For this review, take the finished solid that the model builds, in its own axes (mm). A direction names the side the tool comes from. Give positions to 0.01 mm unless a question says otherwise; leave off trailing zeros. Loops run counter-clockwise (first coordinate to the right, second up) from the corner with the lowest first, then second, coordinate; pieces in that order, holes last.
```python
from build123d import *

# Parameters (mm, degrees)
EXTRUDE_1_DEPTH           = 7.5
SKETCH_2_R                = 11
CUT_EXTRUDE_1_DEPTH       = 6
CUT_EXTRUDE_2_REACH       = 111.663
SKETCH_3_R                = 9.5
CUT_EXTRUDE_3_DEPTH       = 1.5
HOLE_WIZARD_M5_1_D        = 4.2
HOLE_WIZARD_M5_1_DEPTH    = 12.4
HOLE_WIZARD_M5_1_TIP      = 1.2618073
HOLE_WIZARD_1_D           = 5.5
HOLE_WIZARD_1_CBORE_D     = 10
HOLE_WIZARD_1_CBORE_DEPTH = 5.7
HOLE_WIZARD_M3_2_D        = 2.5
CUT_EXTRUDE_START         = -6
SKETCH_17_R               = 11
CUT_EXTRUDE_4_DEPTH       = 6
HOLE_WIZARD_M6_1_D        = 5
HOLE_WIZARD_M6_1_DEPTH    = 15
HOLE_WIZARD_M6_1_TIP      = 1.502151548
CHAMFER_1_SIZE            = 2


with BuildPart() as part:
    # 草图1 → 凸台-拉伸1 (new, symmetric)
    with BuildSketch(Plane(origin=(0, 0, 0), x_dir=(0, 0, -1), z_dir=(1, 0, 0))):
        with BuildLine():
            Line((-10, 101), (-10, 36))
            ThreePointArc((-10, 36), (-12.928932188, 28.928932188), (-20, 26))
            Line((-20, 26), (-40, 26))
            Line((-40, 26), (-40, -101))
            Line((-40, -101), (40, -101))
            Line((40, -101), (40, 101))
            Line((40, 101), (-10, 101))
        make_face()
    extrude(amount=EXTRUDE_1_DEPTH, both=True)

    # 草图2 → 切除-拉伸1 (cut)
    with BuildSketch(Plane.ZY.offset(-7.5)):
        with Locations((-25, 71)):
            Circle(SKETCH_2_R)
    extrude(amount=CUT_EXTRUDE_1_DEPTH, mode=Mode.SUBTRACT)

    # 草图3 → 切除-拉伸2 (cut, up to next)
    with BuildSketch(Plane(origin=(-7.5, 0, 0), x_dir=(0, 0, -1), z_dir=(1, 0, 0)), mode=Mode.PRIVATE) as cut_extrude_2_sk1:
        with Locations(Location((25, 71, 0), (0, 0, 180))):
            Circle(SKETCH_3_R)
    cut_extrude_2_tool1 = extrude(cut_extrude_2_sk1.sketch, amount=CUT_EXTRUDE_2_REACH, mode=Mode.PRIVATE) & part.part
    add(cut_extrude_2_tool1.solids().sort_by_distance((-7.5, 71, -25))[0], mode=Mode.SUBTRACT)

    # 草图6 → 切除-拉伸3 (cut)
    with BuildSketch(Plane(origin=(7.5, 0, 0), x_dir=(0, 0, -1), z_dir=(1, 0, 0))):
        with BuildLine():
            Line((-5.5, 101), (3.5, 101))
            Line((3.5, 101), (3.5, -3.25))
            ThreePointArc((3.5, -3.25), (4.030330086, -4.530330086), (2.75, -4))
            Line((2.75, -4), (-4.75, -4))
            ThreePointArc((-4.75, -4), (-6.030330086, -4.530330086), (-5.5, -3.25))
            Line((-5.5, -3.25), (-5.5, 101))
        make_face()
    extrude(amount=-CUT_EXTRUDE_3_DEPTH, mode=Mode.SUBTRACT)

    # M5 螺纹孔1
    with Locations(Plane(origin=(0, -101, 0), x_dir=(-1, 0, 0), z_dir=(0, -1, 0))):
        with Locations((0, 25), (0, -25)):
            Hole(HOLE_WIZARD_M5_1_D / 2, depth=HOLE_WIZARD_M5_1_DEPTH)
            with Locations((0, 0, -(HOLE_WIZARD_M5_1_DEPTH + HOLE_WIZARD_M5_1_TIP / 2))):  # 118° drill point
                Cone(0, HOLE_WIZARD_M5_1_D / 2, HOLE_WIZARD_M5_1_TIP, mode=Mode.SUBTRACT)

    # 打孔尺寸(%根据)内六角圆柱头螺钉的类型1 (through all)
    with Locations(Plane(origin=(7.5, 0, 0), x_dir=(0, 0, -1), z_dir=(1, 0, 0))):
        with Locations((30, 4), (-30, 4)):
            CounterBoreHole(HOLE_WIZARD_1_D / 2, HOLE_WIZARD_1_CBORE_D / 2, HOLE_WIZARD_1_CBORE_DEPTH)

    # M3 螺纹孔2 (through all)
    with Locations(Plane(origin=(6, 0, 0), x_dir=(0, 0, -1), z_dir=(1, 0, 0))):
        with Locations((-1, 91), (-1, 71), (-1, 51), (-1, 31), (-1, 11)):
            Hole(HOLE_WIZARD_M3_2_D / 2)

    # 草图17 → 切除-拉伸4 (cut)
    with BuildSketch(Plane.ZY.offset(7.5).offset(CUT_EXTRUDE_START)):
        with Locations((-25, 71)):
            Circle(SKETCH_17_R)
    extrude(amount=CUT_EXTRUDE_4_DEPTH, mode=Mode.SUBTRACT)

    # M6 螺纹孔1
    with Locations(Plane(origin=(0, 0, -40), x_dir=(-1, 0, 0), z_dir=(0, 0, -1))):
        with Locations((0, 51), (0, 91)):
            Hole(HOLE_WIZARD_M6_1_D / 2, depth=HOLE_WIZARD_M6_1_DEPTH)
            with Locations((0, 0, -(HOLE_WIZARD_M6_1_DEPTH + HOLE_WIZARD_M6_1_TIP / 2))):  # 118° drill point
                Cone(0, HOLE_WIZARD_M6_1_D / 2, HOLE_WIZARD_M6_1_TIP, mode=Mode.SUBTRACT)

    # 倒角1
    chamfer_1_edges = [part.edges().sort_by_distance(p)[0] for p in [
        (0, 26, 40),
        (0, 101, 10),
        (0, 101, -40),
    ]]
    chamfer(chamfer_1_edges, length=CHAMFER_1_SIZE)


solid = part.part
```
Item 1: Tool access review of faces 1 (the cylindrical face through (5, 4, -25)), 2 (the cylindrical face through (1.13, -94.71, -26.77)), 3 (the cylindrical face through (-0.33, 93.48, -32.39)): name each direction out of +Z, -Z, +X, -X, +Y, -Y from which nothing blocks a thin tool from reaching the whole face with its end or side.
Answer:
face 1: +X
face 2: -Y
face 3: -Z
Item 2: For L1, parallel to Z at x = 0, y = -93.5; L2, parallel to Y at x = 2.75, z = 1; L3, parallel to X at y = 51, z = -30.75, list the stretches that pass through material, from the lowest coordinate up.
Answer:
L1: z = -40 to -27.1, -22.9 to 22.9, 27.1 to 40
L2: y = -101 to 9.75, 12.25 to 29.75, 32.25 to 49.75, 52.25 to 69.75, 72.25 to 89.75, 92.25 to 101
L3: x = -7.5 to -2.5, 2.5 to 7.5
Item 3: Take a section at C-C on y = 45. Give the boundary of the cut face in (x, z), and give its area (4 significant figures).
Answer:
outline: (-7.5, -40) - (7.5, -40) - (7.5, -3.5) - (6, -3.5) - (6, 5.5) - (7.5, 5.5) - (7.5, 10) - (-7.5, 10) - close
area: 736.5 mm2
Item 4: Take a section at D-D on z = 13. Give the boundary of the cut face in (x, y).
Answer:
outline: (-7.5, -101) - (7.5, -101) - (7.5, 28.86) - (-7.5, 28.86) - close
Item 5: Take a section at B-B on x = -5.5. State how many separate pieces and enclosed holes the cut face has, and give its area (3 significant figures).
Answer:
separate pieces: 1
enclosed holes: 8
area: 13,500 mm2
Item 6: Take a section at A-A on z = 30. Give the boundary of the cut face in (x, y), and give its area (3 significant figures).
Answer:
outline: (-7.5, -101) - (7.5, -101) - (7.5, -1) - (1.8, -1) - (1.8, 1.25) - (-7.5, 1.25) - close; (-7.5, 6.75) - (1.8, 6.75) - (1.8, 9) - (7.5, 9) - (7.5, 26) - (-7.5, 26) - close
area: 1,800 mm2
Item 7: The part is to be moulded in two halves that separate along X. For faces 4 (the flat face through (0, 68, 10)), 5 (the flat face through (7.5, -21, 1)), 6 (the conical face through (0.06, 51.43, -23.76)), say which applies: released by +X, released by -X, zero draft, split by the parting line, or undercut.
Answer:
face 4: zero draft
face 5: released by +X
face 6: undercut
Item 8: Clearance check with flat-ended pins moving along their axes: pin 1 Ø3 at (y, z) = (71, 1) entering from +X; pin 2 Ø3 at (y, z) = (5.5, 32) entering from +X; pin 3 Ø2 at (y, z) = (91, 1) entering from -X; pin 4 Ø7.5 at (x, y) = (1, 76.5) entering from +Z. State where each tip first meets the part, or that it passes through.
Answer:
pin 1: stops at x = 6
pin 2: stops at x = 1.8
pin 3: passes through
pin 4: stops at z = 10
